from build123d import *

# Parameters (mm, degrees)
SKETCH1_W           = 280
SKETCH1_H           = 255
SKETCH1_R           = 3.5
BOSS_EXTRUDE1_DEPTH = 14
SKETCH6_W           = 70
SKETCH6_H           = 255
CUT_EXTRUDE3_DEPTH  = 2


with BuildPart() as part:
    # Sketch1 → Boss-Extrude1 (new body)
    with BuildSketch(Plane(origin=(0, 0, 0), x_dir=(0, 0, -1), z_dir=(1, 0, 0))):
        Rectangle(SKETCH1_W, SKETCH1_H)
        with Locations((-120.5, 97.5)):
            Circle(SKETCH1_R, mode=Mode.SUBTRACT)
        with Locations((-85.5, 97.5)):
            Circle(SKETCH1_R, mode=Mode.SUBTRACT)
        with Locations((-120.5, -97.5)):
            Circle(SKETCH1_R, mode=Mode.SUBTRACT)
        with Locations((-85.5, -97.5)):
            Circle(SKETCH1_R, mode=Mode.SUBTRACT)
        with Locations((-120.5, 62.5)):
            Circle(SKETCH1_R, mode=Mode.SUBTRACT)
        with Locations((-85.5, 62.5)):
            Circle(SKETCH1_R, mode=Mode.SUBTRACT)
        with Locations((-120.5, -62.5)):
            Circle(SKETCH1_R, mode=Mode.SUBTRACT)
        with Locations((-85.5, -62.5)):
            Circle(SKETCH1_R, mode=Mode.SUBTRACT)
        with Locations((85.5, 97.5)):
            Circle(SKETCH1_R, mode=Mode.SUBTRACT)
        with Locations((120.5, 97.5)):
            Circle(SKETCH1_R, mode=Mode.SUBTRACT)
        with Locations((85.5, -62.5)):
            Circle(SKETCH1_R, mode=Mode.SUBTRACT)
        with Locations((120.5, -62.5)):
            Circle(SKETCH1_R, mode=Mode.SUBTRACT)
        with Locations((85.5, -97.5)):
            Circle(SKETCH1_R, mode=Mode.SUBTRACT)
        with Locations((120.5, -97.5)):
            Circle(SKETCH1_R, mode=Mode.SUBTRACT)
        with Locations((85.5, 62.5)):
            Circle(SKETCH1_R, mode=Mode.SUBTRACT)
        with Locations((120.5, 62.5)):
            Circle(SKETCH1_R, mode=Mode.SUBTRACT)
    extrude(amount=BOSS_EXTRUDE1_DEPTH)

    # Sketch6 → Cut-Extrude3 (cut)
    with BuildSketch(Plane.ZY):
        with Locations((-105, 0)):
            Rectangle(SKETCH6_W, SKETCH6_H)
        with Locations((105, 0)):
            Rectangle(SKETCH6_W, SKETCH6_H)
    extrude(amount=-CUT_EXTRUDE3_DEPTH, mode=Mode.SUBTRACT)


solid = part.part
Read the model definition and answer for the solid it produces. Units are mm, in the model's axes. A direction names the side the tool comes from. Give positions to 0.01 mm unless a question says otherwise; leave off trailing zeros. Write each loop counter-clockwise with the first axis right and the second up, starting at its lowest first coordinate (ties: lowest second). Pieces come first, ordered by that corner, then holes. Notation, with made-up numbers: M -27,0 L 9,0 A17 cw 9,12 Z; hole C -37.5,-10.5 d5. An arc over 180 degrees is marked long. One line per item, written item: value. Start each with the question number.
(1) A tool of negligible diameter and unlimited length cuts with its end or side. For faces 1 (the flat face through (2, 2, -105)), 2 (the flat face through (7, 127.5, 2)), from which of +Z, -Z, +X, -X, +Y, -Y can it reach the whole face along a straight path? Write none if from no direction.
(2) Determine the mould class of faces 3 (the cylindrical face through (7.916, -63.841, 82.267)), 4 (the flat face through (8, -2, 140)), 5 (the flat face through (8, -2, -140)) for opening direction Z: pulls with the +Z half, pulls with the -Z half, needs draft (parallel to the pull), parting line crosses it, or undercut.
(3) Find section A-A (y = -62.5). Determine the outline of the cut face in (x, z).
(4) Find section C-C (y = 12). Determine the outline of the cut face in (x, z), plus the area to 3 significant figures.
(5) Find section B-B (z = 85.5). Determine the outline of the cut face in (x, y).
(6) Find the intervals of material crossed by line 1 (Z direction, x = 6.25, y = 62.5); line 2 (Y direction, x = 6, z = 85.5); line 3 (Y direction, x = 6.5, z = 83), in increasing order.
(7) Flat-ended cylindrical pins translate along their axes: pin 1 Ø4 at (y, z) = (-62.5, 120.5) entering from -X; pin 2 Ø9 at (y, z) = (-97.5, -120.5) entering from -X; pin 3 Ø0.6 at (x, y) = (1.5, -20.5) entering from +Z; pin 4 Ø0.6 at (x, y) = (1, -59) entering from -Z. Find the tip coordinate at first contact, or state that the pin passes through.
Results below:
1. face 1: -Z, -X, +Y, -Y
1. face 2: +Z, -Z, +X, -X, +Y
2. face 3: undercut
2. face 4: pulls with the +Z half
2. face 5: pulls with the -Z half
3. outline: M 0,-70 L 2,-70 L 2,-82 L 14,-82 L 14,82 L 2,82 L 2,70 L 0,70 Z; M 2,-140 L 14,-140 L 14,-124 L 2,-124 Z; M 2,-117 L 14,-117 L 14,-89 L 2,-89 Z; M 2,89 L 14,89 L 14,117 L 2,117 Z; M 2,124 L 14,124 L 14,140 L 2,140 Z
4. outline: M 0,-70 L 2,-70 L 2,-140 L 14,-140 L 14,140 L 2,140 L 2,70 L 0,70 Z
4. area: 3,640 mm^2
5. outline: M 2,-127.5 L 14,-127.5 L 14,-101 L 2,-101 Z; M 2,-94 L 14,-94 L 14,-66 L 2,-66 Z; M 2,-59 L 14,-59 L 14,59 L 2,59 Z; M 2,66 L 14,66 L 14,94 L 2,94 Z; M 2,101 L 14,101 L 14,127.5 L 2,127.5 Z
6. line 1: z = -140 to -124, -117 to -89, -82 to 82, 89 to 117, 124 to 140
6. line 2: y = -127.5 to -101, -94 to -66, -59 to 59, 66 to 94, 101 to 127.5
6. line 3: y = -127.5 to -99.95, -95.05 to -64.95, -60.05 to 60.05, 64.95 to 95.05, 99.95 to 127.5
7. pin 1: passes through
7. pin 2: stops at x = 2
7. pin 3: stops at z = 70
7. pin 4: stops at z = -70
